Design review of the part built by this model. Coordinates are the model's own, in mm. A direction names the side the tool comes from. Coordinates: 2 decimals unless noted, no trailing zeros. Loops run counter-clockwise (first coordinate to the right, second up) from the corner with the lowest first, then second, coordinate; pieces in that order, holes last. Notation, with made-up numbers: (-10, 69) -> (18, 69) arc R18 ccw to (18, 87) -> close; hole circle Ø3 at (27.25, -12). An arc over 180 degrees is marked (long way). Answer in a Markdown table with one row per item.
```python
from build123d import *

# Parameters (mm, degrees)
GBT706_2008_050_5_1_DEPTH = 783.5
CUT_EXTRUDE_1_DEPTH       = 399.080472392


with BuildPart() as part:
    # Sketch1 → Gbt706-2008 热轧等边角钢 050×5(1) (new body)
    with BuildSketch(Plane(origin=(391.75, 0, 0), x_dir=(0, -1, 0), z_dir=(-1, 0, 0))):
        with BuildLine():
            Line((0, 0), (0, 50))
            Line((0, 50), (3.333333333, 50))
            ThreePointArc((3.333333333, 50), (4.511844635, 49.511844635), (5, 48.333333333))
            Line((5, 48.333333333), (5, 10.5))
            ThreePointArc((5, 10.5), (6.610912703, 6.610912703), (10.5, 5))
            Line((10.5, 5), (48.333333333, 5))
            ThreePointArc((48.333333333, 5), (49.511844635, 4.511844635), (50, 3.333333333))
            Line((50, 3.333333333), (50, 0))
            Line((50, 0), (0, 0))
        make_face()
    extrude(amount=GBT706_2008_050_5_1_DEPTH)

    # 草图2 → 切除-拉伸1 (cut, through all)
    with BuildSketch(Plane(origin=(0, 0, 0), x_dir=(1, 0, 0), z_dir=(0, 1, 0))):
        Polygon((-335.25, 0), (-335.25, -7.501394609), (-339.727357684, -7.501394609), (-382.795284633, -12.028016136), (-391.75, -21.973235089), (-391.75, -52.501394609), (-406.75, -52.501394609), (-406.75, 7.498605391), (-335.25, 7.498605391), align=None)
    extrude(amount=-CUT_EXTRUDE_1_DEPTH, mode=Mode.SUBTRACT)


solid = part.part
```
(1) Take a section at C-C on z = 37. Give the boundary of the cut face in (x, y).
Evaluation:
| item | result |
|---|---|
| outline | (-391.75, -5) -> (391.75, -5) -> (391.75, 0) -> (-391.75, 0) -> close |
(2) For pin 1 (3 mm diameter, centred on x = 198.5, y = -37.5, fed in from +Z); pin 2 (10 mm diameter, centred on x = -130.5, z = 36.5, fed in from -Y); pin 3 (5 mm diameter, centred on x = 268, y = -8, fed in from +Z), all flat-tipped, find the tip position at first contact; note any pin that passes through.
Evaluation:
| item | result |
|---|---|
| pin 1 | stops at z = 5 |
| pin 2 | stops at y = -5 |
| pin 3 | stops at z = 8.21 |
(3) Take a section at B-B on y = -24.5. Give the boundary of the cut face in (x, z).
Evaluation:
| item | result |
|---|---|
| outline | (-335.25, 0) -> (391.75, 0) -> (391.75, 5) -> (-335.25, 5) -> close |
(4) To check wall thickness, follow probe 1 along Z at (x, y) = (270.5, -44); probe 2 along Y at (x, z) = (-284.5, 32.5); probe 3 along X at (y, z) = (-33.5, 4.5). State the ranges of each line that lie inside material, in increasing order.
Evaluation:
| item | result |
|---|---|
| probe 1 | z = 0 to 5 |
| probe 2 | y = -5 to 0 |
| probe 3 | x = -335.25 to 391.75 |
(5) Take a section at A-A on x = 190. Give the boundary of the cut face in (y, z).
Evaluation:
| item | result |
|---|---|
| outline | (-50, 0) -> (0, 0) -> (0, 50) -> (-3.33, 50) arc R1.67 ccw to (-5, 48.33) -> (-5, 10.5) arc R5.5 cw to (-10.5, 5) -> (-48.33, 5) arc R1.67 ccw to (-50, 3.33) -> close |
(6) Tool access review of faces 1 (the flat face through (5, -5, 30)), 2 (the flat face through (391.75, -15.9, 4.7)): name each direction out of +Z, -Z, +X, -X, +Y, -Y from which nothing blocks a thin tool from reaching the whole face with its end or side.
Evaluation:
| item | result |
|---|---|
| face 1 | +Z, +X, -X, -Y |
| face 2 | +Z, -Z, +X, +Y, -Y |
